```python
from build123d import *

# Parameters (mm, degrees)
M8_TAPPED_HOLE1_D     = 6.8
M8_TAPPED_HOLE1_DEPTH = 10.957073895
M8_TAPPED_HOLE1_TIP   = 2.042926105


with BuildPart() as part:
    # Sketch1 → Revolve1 (revolve)
    with BuildSketch(Plane(origin=(0, 0, 0), x_dir=(0, 0, -1), z_dir=(1, 0, 0)), mode=Mode.PRIVATE) as revolve1_sk:
        Polygon((0, 150), (0, 187.5), (30, 187.5), (30, 176), (17, 176), (17, 150), align=None)
    revolve(revolve1_sk.sketch.rotate(Axis((0, 0, 0), (0, 0, -1)), 90), axis=Axis((0, 0, 0), (0, 0, -1)))

    # M8 Tapped Hole1
    with Locations(Plane(origin=(0, 0, -17), x_dir=(-1, 0, 0), z_dir=(0, 0, -1))):
        with Locations((0, 162.5), (95.515103498, 131.465261586), (154.546683898, 50.215261586), (154.546683898, -50.215261586), (95.515103498, -131.465261586), (0, -162.5), (-95.515103498, -131.465261586), (-154.546683898, -50.215261586), (-154.546683898, 50.215261586), (-95.515103498, 131.465261586)):
            Hole(M8_TAPPED_HOLE1_D / 2, depth=M8_TAPPED_HOLE1_DEPTH)
            with Locations((0, 0, -(M8_TAPPED_HOLE1_DEPTH + M8_TAPPED_HOLE1_TIP / 2))):  # 118° drill point
                Cone(0, M8_TAPPED_HOLE1_D / 2, M8_TAPPED_HOLE1_TIP, mode=Mode.SUBTRACT)


solid = part.part
```
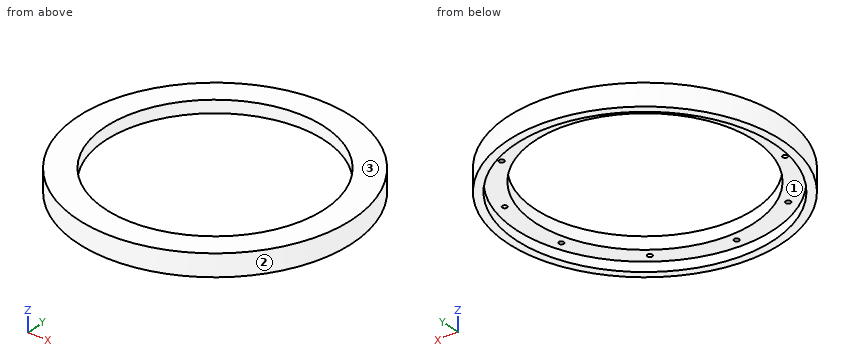
Work out the finished part from the listing and answer in its coordinate system (mm). Face numbers are marked on the shaded views. Round coordinates to 2 decimals unless told otherwise and drop trailing zeros. Order: outer loops, then holes, each group sorted by start corner. A loop starts at its lowest first (then second) coordinate and runs counter-clockwise, first axis right, second up.
Q1. A cutting plane is placed at A-A, the plane y = 0. Determine the outline of the cut face in (x, z).
Solution:
outline: (-187.5, -30) - (-176, -30) - (-176, -17) - (-150, -17) - (-150, 0) - (-187.5, 0) - close; (150, -17) - (176, -17) - (176, -30) - (187.5, -30) - (187.5, 0) - (150, 0) - close
Q2. A cutting plane is placed at B-B, the plane x = 83.5. Determine the outline of the cut face in (y, z), then the cut area to 3 significant figures.
Solution:
outline: (-167.88, -30) - (-154.93, -30) - (-154.93, -17) - (-124.61, -17) - (-124.61, 0) - (-167.88, 0) - close; (124.61, -17) - (154.93, -17) - (154.93, -30) - (167.88, -30) - (167.88, 0) - (124.61, 0) - close
area: 1,810 mm2
Q3. A cutting plane is placed at C-C, the plane z = -11. Count the separate pieces of the cut face and the enclosed holes in it, then the cut area to 3 significant figures.
Solution:
separate pieces: 1
enclosed holes: 11
area: 39,400 mm2
Q4. Given pin 1 Ø1.5 at (y, z) = (-99, -8) entering from -X; pin 2 Ø9 at (x, y) = (95.52, -131.47) entering from +Z; pin 3 Ø4 at (y, z) = (-55.5, -9) entering from +X; pin 4 Ø2 at (y, z) = (-94, -5) entering from -X, each flat-ended and moving along its own axis, determine where each tip first touches the part or whether it passes through.
Solution:
pin 1: stops at x = -159.7
pin 2: stops at z = 0
pin 3: stops at x = 179.71
pin 4: stops at x = -162.81
Q5. The mould has two halves that part along X. Classify the marked faces 1, 2 and 3: pulls with the +X half, pulls with the -X half, needs draft (parallel to the pull), parting line crosses it, or undercut.
Solution:
face 1: undercut
face 2: parting line crosses it
face 3: needs draft
Q6. Find the intervals of material crossed by line 1 along Y through (x, z) = (0, -12); line 2 along Y through (x, z) = (0, -20.5); line 3 along Y through (x, z) = (-85, -3.5), in increasing order.
Solution:
line 1: y = -187.5 to -165.9, -159.1 to -150, 150 to 159.1, 165.9 to 187.5
line 2: y = -187.5 to -176, 176 to 187.5
line 3: y = -167.13 to -123.59, 123.59 to 167.13
